from build123d import *

# Parameters (mm, degrees)
SKETCH1_W             = 60
SKETCH1_H             = 32
BOSS_EXTRUDE1_DEPTH   = 20
SKETCH2_R             = 5
CUT_EXTRUDE1_DEPTH    = 42
CHAMFER1_SIZE         = 3
M6_TAPPED_HOLE1_D     = 5
M6_TAPPED_HOLE1_DEPTH = 15
M6_TAPPED_HOLE1_TIP   = 1.502151548
SKETCH6_W             = 15
SKETCH6_H             = 30
CUT_EXTRUDE2_DEPTH    = 25
FILLET1_R             = 3


with BuildPart() as part:
    # Sketch1 → Boss-Extrude1 (new body)
    with BuildSketch(Plane(origin=(0, 0, 0), x_dir=(1, 0, 0), z_dir=(0, 1, 0))):
        Rectangle(SKETCH1_W, SKETCH1_H)
    extrude(amount=BOSS_EXTRUDE1_DEPTH)

    # Sketch2 → Cut-Extrude1 (cut)
    with BuildSketch(Plane.XY.offset(16)):
        with Locations((20, 10)):
            Circle(SKETCH2_R)
    extrude(amount=-CUT_EXTRUDE1_DEPTH, mode=Mode.SUBTRACT)

    # Chamfer1
    chamfer1_edges = [part.edges().sort_by_distance(p)[0] for p in [
        (30, 20, 0),
        (-30, 20, 0),
        (30, 0, 0),
        (-30, 0, 0),
    ]]
    chamfer(chamfer1_edges, length=CHAMFER1_SIZE)

    # M6 Tapped Hole1
    with Locations(Plane.ZY.offset(30)):
        with Locations((-10, 10), (10, 10)):
            Hole(M6_TAPPED_HOLE1_D / 2, depth=M6_TAPPED_HOLE1_DEPTH)
            with Locations((0, 0, -(M6_TAPPED_HOLE1_DEPTH + M6_TAPPED_HOLE1_TIP / 2))):  # 118° drill point
                Cone(0, M6_TAPPED_HOLE1_D / 2, M6_TAPPED_HOLE1_TIP, mode=Mode.SUBTRACT)

    # Sketch6 → Cut-Extrude2 (cut)
    with BuildSketch(Plane(origin=(30, 0, 0), x_dir=(0, 0, -1), z_dir=(1, 0, 0))):
        with Locations((0, 10)):
            Rectangle(SKETCH6_W, SKETCH6_H)
    extrude(amount=-CUT_EXTRUDE2_DEPTH, mode=Mode.SUBTRACT)

    # Fillet1
    fillet1_edges = [part.edges().sort_by_distance(p)[0] for p in [
        (5, 10, -7.5),
        (5, 10, 7.5),
    ]]
    fillet(fillet1_edges, radius=FILLET1_R)


solid = part.part
The listing builds one solid part. Answer for the finished solid, in the listing's coordinates (mm). A direction names the side the tool comes from. Coordinates: 2 decimals unless noted, no trailing zeros. Loops run counter-clockwise (first coordinate to the right, second up) from the corner with the lowest first, then second, coordinate; pieces in that order, holes last. Notation, with made-up numbers: (-23.75, 3.5) -> (1.25, 3.5) arc R15 ccw to (1.25, 27.5) -> close; hole circle Ø2 at (36.25, 66.25). An arc over 180 degrees is marked (long way). Answer in a Markdown table with one row per item. Add a question column.
1. Flat-ended cylindrical pins translate along their axes: P1, Ø4.5, axis at y = 10, z = -10, coming from the -X side; P2, Ø12, axis at y = 18, z = 1, coming from the +X side; P3, Ø9, axis at x = 20, y = 10, coming from the +Z side; P4, Ø10, axis at y = 9, z = -1.5, coming from the +X side. Find the tip coordinate at first contact, or state that the pin passes through.
2. For faces 4 (the cylindrical face through (19.349, 14.957, -11.69)), 5 (the flat face through (14, 10, -7.5)), 6 (the cylindrical face through (-22.4, 7.56, 10.54)), determine the directions among +Z, -Z, +X, -X, +Y, -Y from which every point of the face is accessible in a straight line to the end or side of a thin tool.
3. Consider line 1 (Z direction, x = -21.5, y = 10); line 2 (Z direction, x = 10.5, y = 13.25); line 3 (Y direction, x = -24, z = -10). Determine where each line is inside the solid, lowest interval first. Write a range as [from, to].
4. The part is cut by section A-A, the plane x = 20. Write down the section's boundary in (y, z).
5. The part is cut by section B-B, the plane y = 13.5. Write down the section's boundary in (x, z).
6. The part is cut by section C-C, the plane x = 6. Write down the section's boundary in (y, z).
7. Determine the mould class of faces 1 (the flat face through (-6, 0, 0)), 2 (the cylindrical face through (19.349, 14.957, 11.81)), 3 (the flat face through (-28, 1, 0)) for opening direction X: +X half, -X half, draft (parallel to the pull), parting line (faces both ways), or undercut.
8. The part is cut by section D-D, the plane y = 4.25. Write down the section's boundary in (x, z).
Answer below:
| question | item | result |
|---|---|---|
| 1 | P1 | x = -14.85 |
| 1 | P2 | x = 6.34 |
| 1 | P3 | through |
| 1 | P4 | x = 5.76 |
| 2 | face 4 | +Z, -Z |
| 2 | face 5 | +X, +Y, -Y |
| 2 | face 6 | -X |
| 3 | line 1 | [-16, -12.5], [-7.5, 7.5], [12.5, 16] |
| 3 | line 2 | [-16, -7.5], [7.5, 16] |
| 3 | line 3 | [0, 7.5], [12.5, 20] |
| 4 | outline | (0, -16) -> (5, -16) -> (5, -7.5) -> (0, -7.5) -> close; (0, 7.5) -> (5, 7.5) -> (5, 16) -> (0, 16) -> close; (15, -16) -> (20, -16) -> (20, -7.5) -> (15, -7.5) -> close; (15, 7.5) -> (20, 7.5) -> (20, 16) -> (15, 16) -> close |
| 5 | outline | (-30, -16) -> (16.43, -16) -> (16.43, -7.5) -> (8, -7.5) arc R3 cw to (5, -4.5) -> (5, 4.5) arc R3 cw to (8, 7.5) -> (16.43, 7.5) -> (16.43, 16) -> (-30, 16) -> close; (23.57, -16) -> (30, -16) -> (30, -7.5) -> (23.57, -7.5) -> close; (23.57, 7.5) -> (30, 7.5) -> (30, 16) -> (23.57, 16) -> close |
| 6 | outline | (0, -16) -> (20, -16) -> (20, -6.74) -> (0, -6.74) -> close; (0, 6.74) -> (20, 6.74) -> (20, 16) -> (0, 16) -> close |
| 7 | face 1 | draft |
| 7 | face 2 | undercut |
| 7 | face 3 | -X half |
| 8 | outline | (-30, -16) -> (30, -16) -> (30, -7.5) -> (8, -7.5) arc R3 cw to (5, -4.5) -> (5, 4.5) arc R3 cw to (8, 7.5) -> (30, 7.5) -> (30, 16) -> (-30, 16) -> close |
